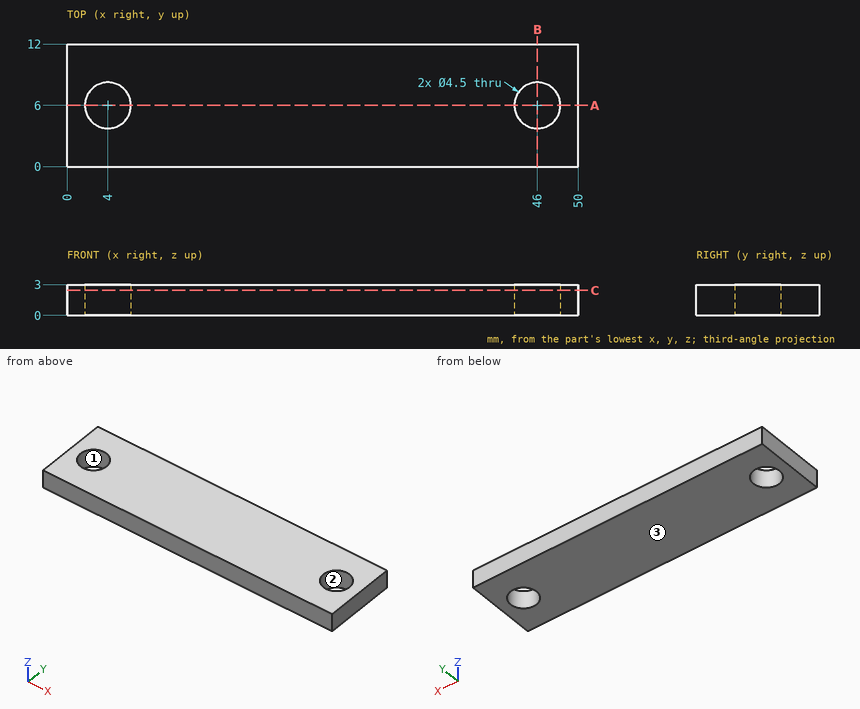
Study the drawing (mm; zero at the part's minimum x, y, z) and answer. Give positions to 0.01 mm unless a question says otherwise; leave off trailing zeros. Order: outer loops, then holes, each group sorted by start corner. A loop starts at its lowest first (then second) coordinate and runs counter-clockwise, first axis right, second up.
1) Determine the mould class of the marked faces 1, 2 and 3 for opening direction Y: pulls with the +Y half, pulls with the -Y half, needs draft (parallel to the pull), parting line crosses it, or undercut.
Reported:
face 1: undercut
face 2: undercut
face 3: needs draft
2) Find section C-C on z = 2.45. Write down the section's boundary in (x, y).
Reported:
outline: (0, 0) - (50, 0) - (50, 12) - (0, 12) - close; hole circle Ø4.5 at (4, 6); hole circle Ø4.5 at (46, 6)
3) Consider line 1 along X through (y, z) = (7, 2.3); line 2 along Y through (x, z) = (4, 0.8); line 3 along X through (y, z) = (8, 1.2). Determine where each line is inside the solid, lowest interval first.
Reported:
line 1: x = 0 to 1.98, 6.02 to 43.98, 48.02 to 50
line 2: y = 0 to 3.75, 8.25 to 12
line 3: x = 0 to 2.97, 5.03 to 44.97, 47.03 to 50
4) Find section B-B on x = 46. Write down the section's boundary in (y, z), then the cut area to 3 significant figures.
Reported:
outline: (0, 0) - (3.75, 0) - (3.75, 3) - (0, 3) - close; (8.25, 0) - (12, 0) - (12, 3) - (8.25, 3) - close
area: 22.5 mm2
5) Find section A-A on y = 6. Write down the section's boundary in (x, z).
Reported:
outline: (0, 0) - (1.75, 0) - (1.75, 3) - (0, 3) - close; (6.25, 0) - (43.75, 0) - (43.75, 3) - (6.25, 3) - close; (48.25, 0) - (50, 0) - (50, 3) - (48.25, 3) - close
